from build123d import *

# Parameters (mm, degrees)
SKETCH1_R           = 17
SKETCH1_R_2         = 12.75
BOSS_EXTRUDE1_DEPTH = 4
CHAMFER1_SIZE       = 0.2


with BuildPart() as part:
    # Sketch1 → Boss-Extrude1 (new, symmetric)
    with BuildSketch(Plane(origin=(0, 0, 0), x_dir=(0, 0, -1), z_dir=(1, 0, 0))):
        Circle(SKETCH1_R)
        Circle(SKETCH1_R_2, mode=Mode.SUBTRACT)
    extrude(amount=BOSS_EXTRUDE1_DEPTH, both=True)

    # Chamfer1
    chamfer1_edges = [part.edges().sort_by_distance(p)[0] for p in [
        (-4, 0, 17),
        (4, 0, 17),
        (-4, 0, 12.75),
        (4, 0, 12.75),
    ]]
    chamfer(chamfer1_edges, length=CHAMFER1_SIZE)


solid = part.part
Source: CAD feature listing. Evaluate the final solid. Frame: model axes, mm. Give positions to 0.01 mm unless a question says otherwise; leave off trailing zeros. Write each loop counter-clockwise with the first axis right and the second up, starting at its lowest first coordinate (ties: lowest second). Pieces come first, ordered by that corner, then holes. Notation, with made-up numbers: M -0.5,74 L 28.5,74 A18 cw 28.5,88 Z; hole C 83,-21 d7. An arc over 180 degrees is marked long. Return JSON: item names as keys, results as strings. Group by question number.
1) Cut plane C-C, the plane x = 0.25. Output: boundary loops of the cut face in (y, z).
2) Draft query along Z for faces 1 (the face through (4, -10, -9)), 2 (the face through (-0.053, -12.447, 2.764)), 3 (the face through (0.053, 14.334, -9.139)). Return one class per face: released by +Z, released by -Z, zero draft, split by the parting line, or undercut.
3) Ray query, L1, parallel to Y at x = -0.5, z = 0; L2, parallel to Z at x = 0.75, y = -7; L3, parallel to Y at x = 3.25, z = -9. Return the intervals inside material, ascending.
4) Cut plane A-A, the plane z = 0. Output: boundary loops of the cut face in (x, y).
5) First-contact query: pin 1 Ø3 at (x, z) = (-2, -5.5) entering from +Y; pin 2 Ø3 at (x, z) = (-3, 6) entering from +Y; pin 3 Ø1 at (x, y) = (-2.5, -10) entering from -Z. Flat tips, straight axial feed; report the tip coordinate or a pass-through.
Data:
{
 "1": {"outline": "C 0,0 d34; hole C 0,0 d25.5"},
 "2": {"face 1": "zero draft", "face 2": "undercut", "face 3": "split by the parting line"},
 "3": {"L1": "y = -17 to -12.75, 12.75 to 17", "L2": "z = -15.49 to -10.66, 10.66 to 15.49", "L3": "y = -14.42 to -9.03, 9.03 to 14.42"},
 "4": {"outline": "M -4,-16.8 L -3.8,-17 L 3.8,-17 L 4,-16.8 L 4,-12.95 L 3.8,-12.75 L -3.8,-12.75 L -4,-12.95 Z; M -4,12.95 L -3.8,12.75 L 3.8,12.75 L 4,12.95 L 4,16.8 L 3.8,17 L -3.8,17 L -4,16.8 Z"},
 "5": {"pin 1": "stops at y = 16.52", "pin 2": "stops at y = 16.39", "pin 3": "stops at z = -14.1"}
}
